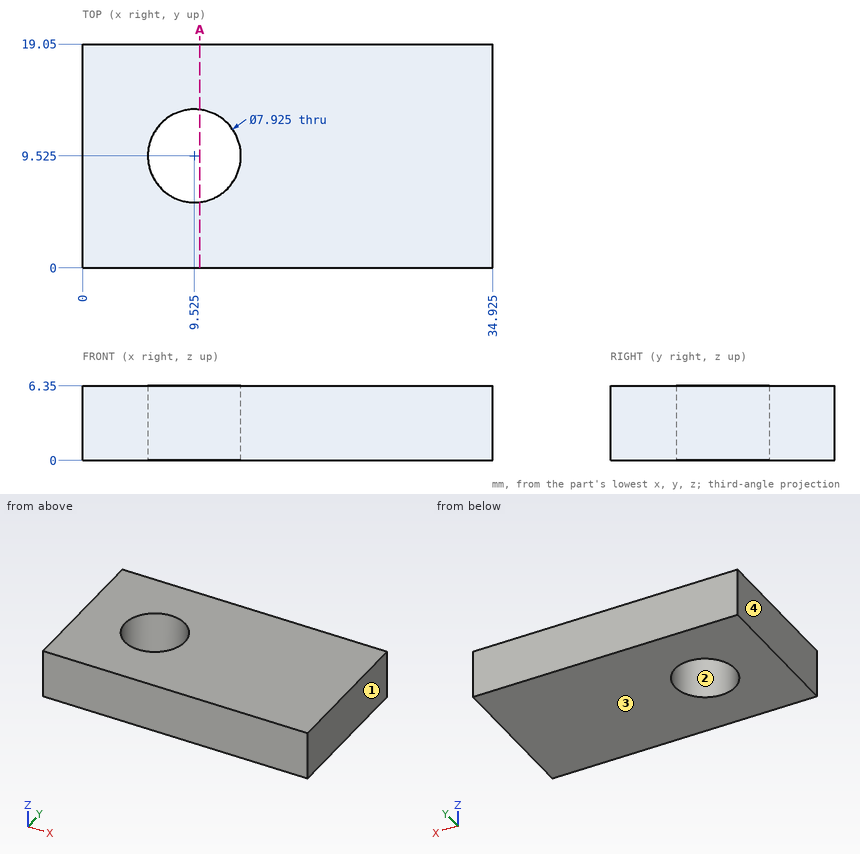
Geometry check sheet. Reference: drawing and pictorial views, mm from the part's lowest x, y, z. Give positions to 0.01 mm unless a question says otherwise; leave off trailing zeros. Order: outer loops, then holes, each group sorted by start corner. A loop starts at its lowest first (then second) coordinate and runs counter-clockwise, first axis right, second up. Notation, with made-up numbers: (6.25, 4) -> (54.25, 4) arc R23 ccw to (54.25, 36) -> close; hole circle Ø9 at (46, -27). An arc over 180 degrees is marked (long way). Use CSV: the item, a comma, the result in double quotes. Start each with the question number.
1) Sectioned sample at A-A, the plane x = 10. Record the boundary of the cut face in (y, z), plus the area to 3 significant figures.
2) Go/stop test with a flat-tipped pin: P1, Ø5, axis at x = 9.525, y = 9.525, coming from the -Z side. Record where the tip stops, or that it passes through.
3) Mould release check, pull along X, two halves, no side actions. Record for the marked faces 1, 2, 3 and 4: released by +X, released by -X, zero draft, split by the parting line, or undercut.
4) Material ranges on line 1 (X direction, y = 6.25, z = 0.75) (1 decimal); line 2 (X direction, y = 11.5, z = 3.5) (1 decimal); line 3 (Y direction, x = 13, z = 2.5), recorded low to high. Write a range as from..to.
Recorded:
1,outline,"(0, 0) -> (5.59, 0) -> (5.59, 6.35) -> (0, 6.35) -> close; (13.46, 0) -> (19.05, 0) -> (19.05, 6.35) -> (13.46, 6.35) -> close"
1,area,"71.0 mm2"
2,P1,"through"
3,face 1,"released by +X"
3,face 2,"undercut"
3,face 3,"zero draft"
3,face 4,"released by -X"
4,line 1,"0..7.3, 11.8..34.9"
4,line 2,"0..6.1, 13..34.9"
4,line 3,"0..7.62, 11.43..19.05"
